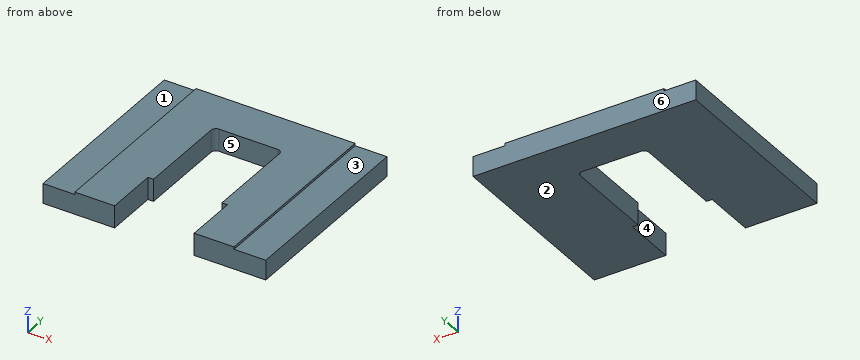
```python
from build123d import *

# Parameters (mm, degrees)
SKETCH_1_W                      = 140
SKETCH_1_H                      = 120
EXTRUDE_1_DEPTH                 = 14
SKETCH_2_W                      = 20
SKETCH_2_H                      = 120
CUT_EXTRUDE_1_DEPTH             = 1.5
CUT_EXTRUDE_2_REACH             = 95.252
SKETCH_3_W                      = 50
SKETCH_3_H                      = 33
CUT_EXTRUDE_3_REACH             = 95.252
SKETCH_4_W                      = 43
SKETCH_4_H                      = 60
CUT_EXTRUDE_3_DIRECTION_2_DEPTH = 94.252345815
FILLET_1_R                      = 3


with BuildPart() as part:
    # 草图1 → 凸台-拉伸1 (new body)
    with BuildSketch(Plane.XY):
        Rectangle(SKETCH_1_W, SKETCH_1_H)
    extrude(amount=EXTRUDE_1_DEPTH)

    # 草图2 → 切除-拉伸1 (cut)
    with BuildSketch(Plane.XY.offset(14)):
        with Locations((-60, 0)):
            Rectangle(SKETCH_2_W, SKETCH_2_H)
        with Locations((60, 0)):
            Rectangle(SKETCH_2_W, SKETCH_2_H)
    extrude(amount=-CUT_EXTRUDE_1_DEPTH, mode=Mode.SUBTRACT)

    # 草图3 → 切除-拉伸2 (cut, up to next)
    with BuildSketch(Plane.XY.offset(14), mode=Mode.PRIVATE) as cut_extrude_2_sk1:
        with Locations((0, -43.5)):
            Rectangle(SKETCH_3_W, SKETCH_3_H)
    cut_extrude_2_tool1 = extrude(cut_extrude_2_sk1.sketch, amount=-CUT_EXTRUDE_2_REACH, mode=Mode.PRIVATE) & part.part
    add(cut_extrude_2_tool1.solids().sort_by_distance((0, -43.5, 14))[0], mode=Mode.SUBTRACT)

    # 草图4 → 切除-拉伸3 (cut, up to next)
    with BuildSketch(Plane(origin=(0, 0, 0), x_dir=(-1, 0, 0), z_dir=(0, 0, -1)), mode=Mode.PRIVATE) as cut_extrude_3_sk1:
        with Locations((0, 3)):
            Rectangle(SKETCH_4_W, SKETCH_4_H)
    cut_extrude_3_tool1 = extrude(cut_extrude_3_sk1.sketch, amount=-CUT_EXTRUDE_3_REACH, mode=Mode.PRIVATE) & part.part
    add(cut_extrude_3_tool1.solids().sort_by_distance((0, 3, 0))[0], mode=Mode.SUBTRACT)

    # 草图4 → 切除-拉伸3 direction 2 (cut)
    with BuildSketch(Plane(origin=(0, 0, 0), x_dir=(-1, 0, 0), z_dir=(0, 0, -1))):
        with Locations((0, 3)):
            Rectangle(SKETCH_4_W, SKETCH_4_H)
    extrude(amount=CUT_EXTRUDE_3_DIRECTION_2_DEPTH, mode=Mode.SUBTRACT)

    # 圆角1
    fillet_1_edges = [part.edges().sort_by_distance(p)[0] for p in [
        (-21.5, 33, 7),
        (21.5, 33, 7),
    ]]
    fillet(fillet_1_edges, radius=FILLET_1_R)


solid = part.part
```
Can you work these out from the model? Positions are in its coordinate system, mm. Face numbers are marked on the shaded views. A direction names the side the tool comes from. Give positions to 0.01 mm unless a question says otherwise; leave off trailing zeros. Loops run counter-clockwise (first coordinate to the right, second up) from the corner with the lowest first, then second, coordinate; pieces in that order, holes last. Notation, with made-up numbers: M -25,-27.75 L -9,-27.75 A14 cw -9,-23.75 Z; hole C 2.5,34 d1. An arc over 180 degrees is marked long. Use CSV: the item, a comma, the result in double quotes. Start each with the question number.
1. Imagine slicing it at D-D, the plane y = -11. Write out the boundary of the cut face in (x, z).
2. For P1, Ø4, axis at x = 7.5, z = 4.5, coming from the -Y side; P2, Ø1.8, axis at x = -23.5, z = 6.5, coming from the -Y side; P3, Ø1.6, axis at y = -2, z = 13.5, coming from the -X side, each with a flat end and sliding along its axis, tell me the tip position at first contact or that it passes through.
3. If I drill on L1, parallel to X at y = -7.5, z = 3.25; L2, parallel to X at y = -31, z = 10; L3, parallel to Y at x = -23.5, z = 3.75, over which ranges is the centre line in solid material (lowest first)?
4. Imagine slicing it at B-B, the plane y = 46. Write out the boundary of the cut face in (x, z).
5. If we mould it in two halves opening along X, with no side actions, what happens to the marked faces 5 and 6? For each: released by +X, released by -X, zero draft, split by the parting line, or undercut.
6. Imagine slicing it at C-C, the plane z = 6.25. Write out the boundary of the cut face in (x, y).
7. On a 3-axis mill with a long thin cutter (end or side, diameter ignored), from which of +Z, -Z, +X, -X, +Y, -Y can I reach the whole of each face in a straight line? I mean the marked faces 1, 2, 3 and 4. Say none if no direction works.
8. Imagine slicing it at A-A, the plane y = -36. Write out the boundary of the cut face in (x, z).
Response values:
1,outline,"M -70,0 L -21.5,0 L -21.5,14 L -50,14 L -50,12.5 L -70,12.5 Z; M 21.5,0 L 70,0 L 70,12.5 L 50,12.5 L 50,14 L 21.5,14 Z"
2,P1,"y = 33"
2,P2,"y = -27"
2,P3,"x = -50"
3,L1,"-70 to -21.5, 21.5 to 70"
3,L2,"-70 to -25, 25 to 70"
3,L3,"-27 to 60"
4,outline,"M -70,0 L 70,0 L 70,12.5 L 50,12.5 L 50,14 L -50,14 L -50,12.5 L -70,12.5 Z"
5,face 5,"undercut"
5,face 6,"zero draft"
6,outline,"M -70,-60 L -25,-60 L -25,-27 L -21.5,-27 L -21.5,30 A3 cw -18.5,33 L 18.5,33 A3 cw 21.5,30 L 21.5,-27 L 25,-27 L 25,-60 L 70,-60 L 70,60 L -70,60 Z"
7,face 1,"+Z, -X, +Y, -Y"
7,face 2,"-Z, +X, -X, +Y, -Y"
7,face 3,"+Z, +X, +Y, -Y"
7,face 4,"+Z, -Z, -Y"
8,outline,"M -70,0 L -25,0 L -25,14 L -50,14 L -50,12.5 L -70,12.5 Z; M 25,0 L 70,0 L 70,12.5 L 50,12.5 L 50,14 L 25,14 Z"
